Check sheet for the modelled part. Datum: model origin and axes. Units: mm. A direction names the side the tool comes from. Give positions to 0.01 mm unless a question says otherwise; leave off trailing zeros. Write each loop counter-clockwise with the first axis right and the second up, starting at its lowest first coordinate (ties: lowest second). Pieces come first, ordered by that corner, then holes. Notation, with made-up numbers: (44, -4) -> (71, -4) arc R28 cw to (71, 15) -> close; hole circle Ø11 at (-12.75, -8). An arc over 180 degrees is marked (long way). Use a Markdown table: item, result. Add a question column.
1. Gauge pin test, flat ends, axial feed: P1, Ø6, axis at y = -27, z = 3.5, coming from the -X side; P2, Ø5, axis at y = -22.5, z = 2.5, coming from the -X side; P3, Ø4, axis at y = 8, z = 0, coming from the -X side. Record the tip position at first contact, or that the pin passes through.
2. Release check for a two-part mould opening along Y. For faces 1 (the flat face through (3, 31.5, 0)), 2 (the flat face through (173.33, -35.06, 0.14)), 3 (the flat face through (1, -29, -10)) record: released by +Y, released by -Y, zero draft, split by the parting line, or undercut.
3. Cross-section at C-C (y = -5). Enter the section's corners in (x, z).
4. Scan lines: probe 1 along Z at (x, y) = (-126.5, 29.5); probe 2 along Y at (x, z) = (152.5, -2.75); probe 3 along Y at (x, z) = (61, 6). Record each from-to range of solid material in increasing order. Write a range as [from, to].
5. Cross-section at B-B (z = -0.75). Enter the section's corners in (x, y), then the cut area to 3 significant figures.
6. Set-up check for faces 4 (the flat face through (-1, 23, -5)), 5 (the flat face through (-172.838, -35.146, 0.14)), 6 (the cylindrical face through (205.38, 2.21, -7.46)): record each of +Z, -Z, +X, -X, +Y, -Y from which the full face is reachable in a straight line by a thin tool's end or side.
7. Cross-section at A-A (x = 70). Enter the section's corners in (y, z).
from build123d import *

# Parameters (mm, degrees)
BOSS_EXTRUDE1_DEPTH = 10
CUT_EXTRUDE1_DEPTH  = 5


with BuildPart() as part:
    # Sketch2 → Boss-Extrude1 (new, symmetric)
    with BuildSketch(Plane.XY):
        with BuildLine():
            Line((-185, 32.5), (185, 32.5))
            ThreePointArc((185, 32.5), (217.376327688, 2.832561639), (190.643565774, -32.006251973))
            Line((190.643565774, -32.006251973), (155.524931981, -38.198614636))
            Line((155.524931981, -38.198614636), (-155.524931981, -38.198614636))
            Line((-155.524931981, -38.198614636), (-190.643565774, -32.006251973))
            ThreePointArc((-190.643565774, -32.006251973), (-217.376327688, 2.832561639), (-185, 32.5))
        make_face()
        with BuildLine():
            Line((-185, 20.5), (185, 20.5))
            ThreePointArc((185, 20.5), (205.421991311, 1.786692726), (188.559787642, -20.188558937))
            Line((188.559787642, -20.188558937), (154.475068019, -26.198614636))
            Line((154.475068019, -26.198614636), (-154.475068019, -26.198614636))
            Line((-154.475068019, -26.198614636), (-188.559787642, -20.188558937))
            ThreePointArc((-188.559787642, -20.188558937), (-205.421991311, 1.786692726), (-185, 20.5))
        make_face(mode=Mode.SUBTRACT)
    extrude(amount=BOSS_EXTRUDE1_DEPTH, both=True)

    # Sketch8 → Cut-Extrude1 (cut, symmetric)
    with BuildSketch(Plane.XY):
        with BuildLine():
            Line((155.437443318, -37.198614636), (190.469917597, -31.02144422))
            ThreePointArc((190.469917597, -31.02144422), (216.38013299, 2.745405897), (185, 31.5))
            Line((185, 31.5), (-185, 31.5))
            ThreePointArc((-185, 31.5), (-216.38013299, 2.745405897), (-190.469917597, -31.02144422))
            Line((-190.469917597, -31.02144422), (-155.437443318, -37.198614636))
            Line((-155.437443318, -37.198614636), (155.437443318, -37.198614636))
        make_face()
    extrude(amount=CUT_EXTRUDE1_DEPTH, both=True, mode=Mode.SUBTRACT)


solid = part.part
Worked answers:
| question | item | result |
|---|---|---|
| 1 | P1 | stops at x = -206.91 |
| 1 | P2 | stops at x = -210.62 |
| 1 | P3 | stops at x = -216.94 |
| 2 | face 1 | undercut |
| 2 | face 2 | released by -Y |
| 2 | face 3 | zero draft |
| 3 | outline | (-217.11, -10) -> (-204.88, -10) -> (-204.88, -5) -> (-216.1, -5) -> (-216.1, 5) -> (-204.88, 5) -> (-204.88, 10) -> (-217.11, 10) -> close; (204.88, -10) -> (217.11, -10) -> (217.11, 10) -> (204.88, 10) -> (204.88, 5) -> (216.1, 5) -> (216.1, -5) -> (204.88, -5) -> close |
| 4 | probe 1 | z = [-10, -5], [5, 10] |
| 4 | probe 2 | y = [-38.2, -37.2], [31.5, 32.5] |
| 4 | probe 3 | y = [-38.2, -26.2], [20.5, 32.5] |
| 5 | outline | (-190.64, -32.01) -> (-155.52, -38.2) -> (155.52, -38.2) -> (190.64, -32.01) arc R32.5 ccw to (185, 32.5) -> (-185, 32.5) arc R32.5 ccw to start; hole (-190.47, -31.02) -> (-155.44, -37.2) -> (155.44, -37.2) -> (190.47, -31.02) arc R31.5 ccw to (185, 31.5) -> (-185, 31.5) arc R31.5 ccw to start |
| 5 | area | 942 mm² |
| 6 | face 4 | none |
| 6 | face 5 | +Z, -Z, -X, -Y |
| 6 | face 6 | +Z, -Z |
| 7 | outline | (-38.2, -10) -> (-26.2, -10) -> (-26.2, -5) -> (-37.2, -5) -> (-37.2, 5) -> (-26.2, 5) -> (-26.2, 10) -> (-38.2, 10) -> close; (20.5, -10) -> (32.5, -10) -> (32.5, 10) -> (20.5, 10) -> (20.5, 5) -> (31.5, 5) -> (31.5, -5) -> (20.5, -5) -> close |
